Design review of the part shown in the three views and the two pictorial views. Dimensions are in mm from the part's minimum x, y and z. A direction names the side the tool comes from. Coordinates: 2 decimals unless noted, no trailing zeros. Loops run counter-clockwise (first coordinate to the right, second up) from the corner with the lowest first, then second, coordinate; pieces in that order, holes last. Notation, with made-up numbers: (41, -27) -> (69, -27) arc R14 ccw to (69, -7) -> close; hole circle Ø3 at (85, 17). An arc over 180 degrees is marked (long way). Use a Markdown table: item, result. Add a question column.
Q1. Clearance check with flat-ended pins moving along their axes: pin 1 Ø1 at (y, z) = (18, 24) entering from -X; pin 2 Ø3 at (x, z) = (22, 18) entering from -Y; pin 3 Ø16.5 at (y, z) = (15, 15) entering from -X. State where each tip first meets the part, or that it passes through.
Q2. Take a section at B-B on z = 9.25. Write out the cut boundary in (x, y).
Q3. For probe 1 along Z at (x, y) = (25, 54); probe 2 along Y at (x, z) = (7, 12.75); probe 3 along X at (y, z) = (25, 26), list the stretches that pass through material, from the lowest coordinate up.
Q4. Take a section at C-C on y = 19. Write out the cut boundary in (x, z).
Q5. Take a section at D-D on z = 15. Write out the cut boundary in (x, y), plus the area to 3 significant figures.
Q6. For the marked faces 1 and 2, list the 3-axis set-ups (+Z, -Z, +X, -X, +Y, -Y) from which the entire face can be reached by the end or side of a thin tool; tool diameter is ignored.
Q7. Take a section at A-A on x = 25. Write out the cut boundary in (y, z).
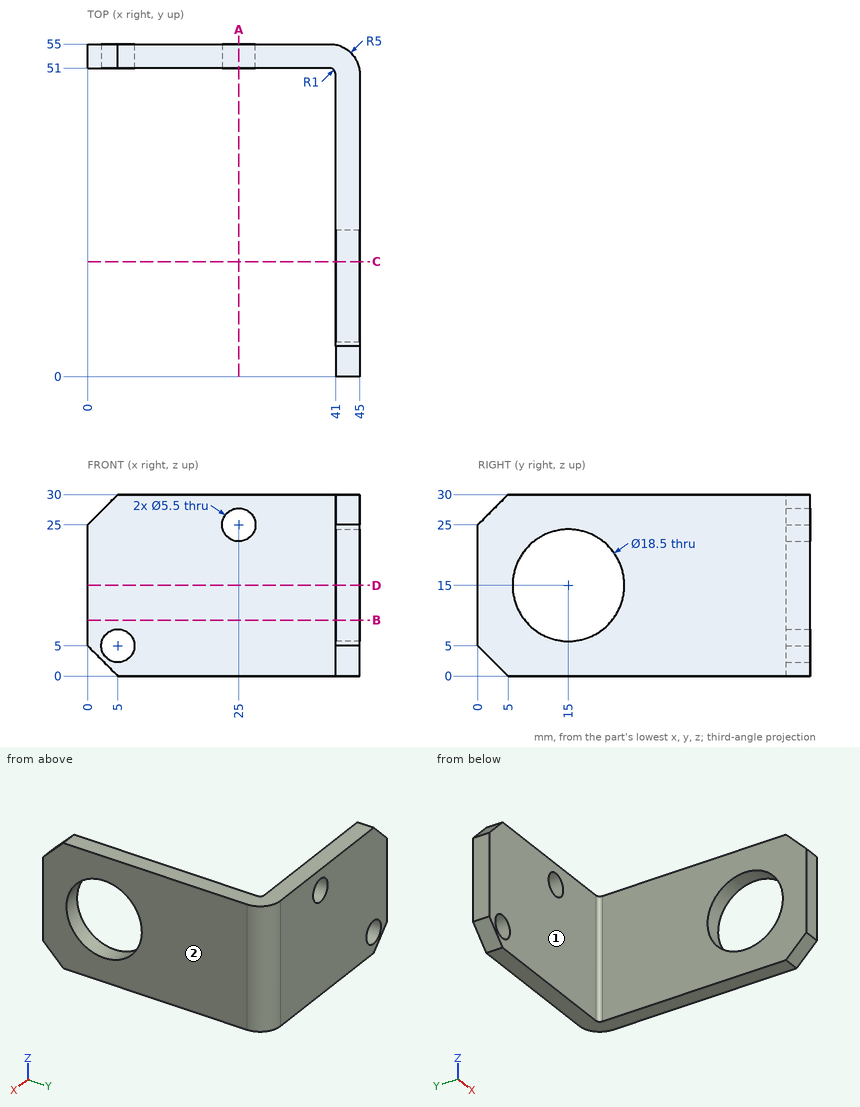
Answer list:
| question | item | result |
|---|---|---|
| 1 | pin 1 | x = 41 |
| 1 | pin 2 | y = 51 |
| 1 | pin 3 | through |
| 2 | outline | (0, 51) -> (40, 51) arc R1 cw to (41, 50) -> (41, 22.25) -> (45, 22.25) -> (45, 50) arc R5 ccw to (40, 55) -> (0, 55) -> close; (41, 0) -> (45, 0) -> (45, 7.75) -> (41, 7.75) -> close |
| 3 | probe 1 | 0 to 22.25, 27.75 to 30 |
| 3 | probe 2 | 51 to 55 |
| 3 | probe 3 | 41 to 45 |
| 4 | outline | (41, 0) -> (45, 0) -> (45, 6.66) -> (41, 6.66) -> close; (41, 23.34) -> (45, 23.34) -> (45, 30) -> (41, 30) -> close |
| 5 | outline | (0, 51) -> (40, 51) arc R1 cw to (41, 50) -> (41, 24.25) -> (45, 24.25) -> (45, 50) arc R5 ccw to (40, 55) -> (0, 55) -> close; (41, 0) -> (45, 0) -> (45, 5.75) -> (41, 5.75) -> close |
| 5 | area | 305 mm² |
| 6 | face 1 | +Z, -Z, -X, -Y |
| 6 | face 2 | +Z, -Z, +X, +Y, -Y |
| 7 | outline | (51, 0) -> (55, 0) -> (55, 22.25) -> (51, 22.25) -> close; (51, 27.75) -> (55, 27.75) -> (55, 30) -> (51, 30) -> close |
